from build123d import *

# Parameters (mm, degrees)
SKETCH1_R           = 30.65
BOSS_EXTRUDE1_DEPTH = 12
SKETCH2_R           = 33.5
BOSS_EXTRUDE2_DEPTH = 3.5
SKETCH3_R           = 24.5
CUT_EXTRUDE1_DEPTH  = 50.847266725
FILLET1_R           = 1
FILLET2_R           = 2
FILLET3_R           = 0.5


with BuildPart() as part:
    # Sketch1 → Boss-Extrude1 (new body)
    with BuildSketch(Plane(origin=(0, 0, 0), x_dir=(1, 0, 0), z_dir=(0, 1, 0))):
        with Locations(Location((0, 0, 0), (0, 0, 270))):
            Circle(SKETCH1_R)
    extrude(amount=-BOSS_EXTRUDE1_DEPTH)

    # Sketch2 → Boss-Extrude2 (add)
    with BuildSketch(Plane(origin=(0, 0, 0), x_dir=(1, 0, 0), z_dir=(0, 1, 0))):
        with Locations(Location((0, 0, 0), (0, 0, 270))):
            Circle(SKETCH2_R)
    extrude(amount=BOSS_EXTRUDE2_DEPTH)

    # Sketch3 → Cut-Extrude1 (cut, through all)
    with BuildSketch(Plane(origin=(0, 3.5, 0), x_dir=(1, 0, 0), z_dir=(0, 1, 0))):
        with Locations(Location((0, 0, 0), (0, 0, 270))):
            Circle(SKETCH3_R)
    extrude(amount=-CUT_EXTRUDE1_DEPTH, mode=Mode.SUBTRACT)

    # Fillet1
    fillet1_edges = [part.edges().sort_by_distance(p)[0] for p in [
        (0, 3.5, -33.5),
    ]]
    fillet(fillet1_edges, radius=FILLET1_R)

    # Fillet2
    fillet2_edges = [part.edges().sort_by_distance(p)[0] for p in [
        (0, -12, -30.65),
    ]]
    fillet(fillet2_edges, radius=FILLET2_R)

    # Fillet3
    fillet3_edges = [part.edges().sort_by_distance(p)[0] for p in [
        (0, -12, -24.5),
        (0, 3.5, -24.5),
        (0, 0, -33.5),
    ]]
    fillet(fillet3_edges, radius=FILLET3_R)


solid = part.part
Model file for the job. Use its own axes, mm. Round coordinates to 2 decimals unless told otherwise and drop trailing zeros. Order: outer loops, then holes, each group sorted by start corner. A loop starts at its lowest first (then second) coordinate and runs counter-clockwise, first axis right, second up. Notation, with made-up numbers: M -3.5,89.5 L 44.5,89.5 A13 cw 44.5,110.5 Z; hole C 54.25,-27.75 d8. An arc over 180 degrees is marked long. Write each question's results on one line, items separated by ' | '. Start each with the question number.
(1) Saw through at B-B, the plane z = 0. Give the cut face in (x, y), then the cut area to 3 significant figures.
(2) Saw through at C-C, the plane y = -1.25. Give the cut face in (x, z).
(3) Drop flat-ended pins along their axis: pin 1 (3 mm diameter, centred on x = -24.5, y = -1, fed in from -Z); pin 2 (1 mm diameter, centred on y = -3, z = 22.5, fed in from +X); pin 3 (5 mm diameter, centred on y = -7, z = -25.5, fed in from -X). Give the stop position or say it passes through.
(4) Probe probe 1 along X at (y, z) = (-3.5, 0); probe 2 along Z at (x, y) = (-22.5, -1.25); probe 3 along Z at (x, y) = (10.5, -4.75). List the from-to ranges inside material, lowest first. Write a range as from..to.
(5) Two-plate mould, pull along Z, no slides. Class faces 1 (the face through (7.36, -4.15, 23.37)), 2 (the face through (30.39, -4.93, -3.99)), 3 (the face through (-22, 0, 22)): pulls with the +Z half, pulls with the -Z half, needs draft (parallel to the pull), parting line crosses it, or undercut.
(6) Saw through at A-A, the plane x = 0. Give the cut face in (y, z), then the cut area to 3 significant figures.
Established:
1) outline: M -33.5,0.5 A0.5 ccw -33,0 L -30.65,0 L -30.65,-10 A2 ccw -28.65,-12 L -25,-12 A0.5 ccw -24.5,-11.5 L -24.5,3 A0.5 ccw -25,3.5 L -32.5,3.5 A1 ccw -33.5,2.5 Z; M 24.5,-11.5 A0.5 ccw 25,-12 L 28.65,-12 A2 ccw 30.65,-10 L 30.65,0 L 33,0 A0.5 ccw 33.5,0.5 L 33.5,2.5 A1 ccw 32.5,3.5 L 25,3.5 A0.5 ccw 24.5,3 Z | area: 208 mm^2
2) outline: C 0,0 d61.3; hole C 0,0 d49
3) pin 1: stops at z = -23.64 | pin 2: stops at x = 21.34 | pin 3: stops at x = -20.26
4) probe 1: x = -30.65..-24.5, 24.5..30.65 | probe 2: z = -20.81..-9.7, 9.7..20.81 | probe 3: z = -28.8..-22.14, 22.14..28.8
5) face 1: undercut | face 2: parting line crosses it | face 3: needs draft
6) outline: M -12,-28.65 A2 ccw -10,-30.65 L 0,-30.65 L 0,-33 A0.5 ccw 0.5,-33.5 L 2.5,-33.5 A1 ccw 3.5,-32.5 L 3.5,-25 A0.5 ccw 3,-24.5 L -11.5,-24.5 A0.5 ccw -12,-25 Z; M -12,25 A0.5 ccw -11.5,24.5 L 3,24.5 A0.5 ccw 3.5,25 L 3.5,32.5 A1 ccw 2.5,33.5 L 0.5,33.5 A0.5 ccw 0,33 L 0,30.65 L -10,30.65 A2 ccw -12,28.65 Z | area: 208 mm^2
